Build history of the part. All positions in model axes, mm. A direction names the side the tool comes from. Give positions to 0.01 mm unless a question says otherwise; leave off trailing zeros. Order: outer loops, then holes, each group sorted by start corner. A loop starts at its lowest first (then second) coordinate and runs counter-clockwise, first axis right, second up. Notation, with made-up numbers: (50, 4.5) -> (81, 4.5) arc R25 cw to (81, 30.5) -> close; hole circle Ø6 at (11.25, -32). An arc over 180 degrees is marked (long way). One line per question, with ' | ' between items. Start each with the question number.
(1) Drill centre lines: L1, parallel to X at y = 7.25, z = 40; L2, parallel to Z at x = -57, y = 4.75; L3, parallel to Z at x = 42.5, y = 6.5. Where is each one in solid material? Low to high. Write a range as from..to.
(2) Cut at C-C (x = 51). Give the cut face in (y, z).
(3) Cut at A-A (z = -38.5). Give the cut face in (x, y), then the cut area to 3 significant figures.
(4) Cut at B-B (y = 3). Give the cut face in (x, z), then the cut area to 3 significant figures.
(5) Which spindle directions (+Z, -Z, +X, -X, +Y, -Y) get a long thin tool onto all of the face, cutting with end or side? Do faces 1 (the face through (82, 7, -82.5)), 2 (the face through (41.43, 7.1, 46)). Say none if no direction does.
from build123d import *

# Parameters (mm, degrees)
SKETCH_1_W          = 200
SKETCH_1_H          = 165
EXTRUDE_1_DEPTH     = 14
CUT_EXTRUDE_1_REACH = 132.393
SKETCH_2_W          = 25
SKETCH_2_H          = 130
FILLET_1_R          = 5


with BuildPart() as part:
    # 草图1 → 凸台-拉伸1 (new body)
    with BuildSketch(Plane(origin=(0, 0, 0), x_dir=(1, 0, 0), z_dir=(0, 1, 0))):
        Rectangle(SKETCH_1_W, SKETCH_1_H)
    extrude(amount=EXTRUDE_1_DEPTH)

    # 草图2 → 切除-拉伸1 (cut, up to next)
    with BuildSketch(Plane.XZ, mode=Mode.PRIVATE) as cut_extrude_1_sk1:
        with Locations((52.5, -17.5)):
            Rectangle(SKETCH_2_W, SKETCH_2_H)
    cut_extrude_1_tool1 = extrude(cut_extrude_1_sk1.sketch, amount=-CUT_EXTRUDE_1_REACH, mode=Mode.PRIVATE) & part.part
    # 草图2 → 切除-拉伸1 (cut, up to next)
    with BuildSketch(Plane.XZ, mode=Mode.PRIVATE) as cut_extrude_1_sk2:
        with Locations((-52.5, -17.5)):
            Rectangle(SKETCH_2_W, SKETCH_2_H)
    cut_extrude_1_tool2 = extrude(cut_extrude_1_sk2.sketch, amount=-CUT_EXTRUDE_1_REACH, mode=Mode.PRIVATE) & part.part
    add(cut_extrude_1_tool1.solids().sort_by_distance((52.5, 0, -17.5))[0], mode=Mode.SUBTRACT)
    add(cut_extrude_1_tool2.solids().sort_by_distance((-52.5, 0, -17.5))[0], mode=Mode.SUBTRACT)

    # 圆角1
    fillet_1_edges = [part.edges().sort_by_distance(p)[0] for p in [
        (40, 7, 47.5),
        (65, 7, 47.5),
        (-40, 7, 47.5),
        (-65, 7, 47.5),
    ]]
    fillet(fillet_1_edges, radius=FILLET_1_R)


solid = part.part
Result set:
1) L1: x = -100..-65, -40..40, 65..100 | L2: z = 47.5..82.5 | L3: z = 46.83..82.5
2) outline: (0, 47.5) -> (14, 47.5) -> (14, 82.5) -> (0, 82.5) -> close
3) outline: (-100, 0) -> (-65, 0) -> (-65, 14) -> (-100, 14) -> close; (-40, 0) -> (40, 0) -> (40, 14) -> (-40, 14) -> close; (65, 0) -> (100, 0) -> (100, 14) -> (65, 14) -> close | area: 2,100 mm2
4) outline: (-100, -82.5) -> (-65, -82.5) -> (-65, 42.5) arc R5 cw to (-60, 47.5) -> (-45, 47.5) arc R5 cw to (-40, 42.5) -> (-40, -82.5) -> (40, -82.5) -> (40, 42.5) arc R5 cw to (45, 47.5) -> (60, 47.5) arc R5 cw to (65, 42.5) -> (65, -82.5) -> (100, -82.5) -> (100, 82.5) -> (-100, 82.5) -> close | area: 26,500 mm2
5) face 1: -Z, +X, -X, +Y, -Y | face 2: -Z, +Y, -Y
